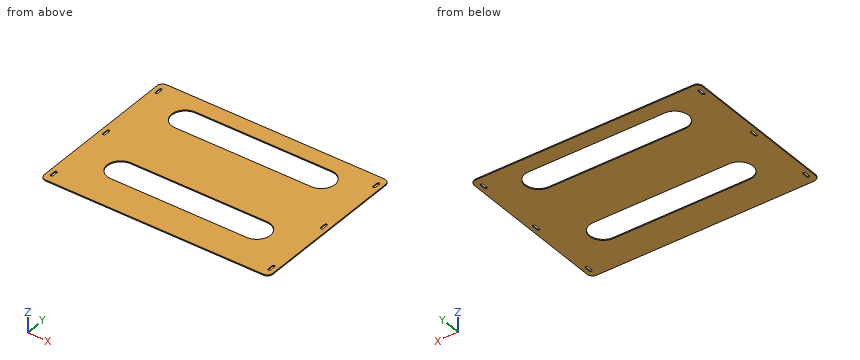
```python
from build123d import *

# Parameters (mm, degrees)
SKETCH_1_W          = 420
SKETCH_1_H          = 300
EXTRUDE_1_DEPTH     = 2
HOLE_WIZARD_M4_2_D  = 3.3
CUT_EXTRUDE_1_DEPTH = 10
FILLET_1_R          = 10
CUT_EXTRUDE_2_DEPTH = 10


with BuildPart() as part:
    # 草图1 → 凸台-拉伸1 (new body)
    with BuildSketch(Plane.XY):
        Rectangle(SKETCH_1_W, SKETCH_1_H)
    extrude(amount=EXTRUDE_1_DEPTH)

    # M4 螺纹孔的螺纹孔钻头2 (through all)
    with Locations(Plane.XY.offset(2)):
        with Locations((200, 0), (-200, -130), (-200, 0), (200, -130)):
            Hole(HOLE_WIZARD_M4_2_D / 2)

    # 草图4 → 切除-拉伸1 (cut)
    with BuildSketch(Plane.XY.offset(2)):
        with BuildLine():
            Line((197.75, -135), (197.75, -125))
            ThreePointArc((197.75, -125), (200, -122.75), (202.25, -125))
            Line((202.25, -125), (202.25, -135))
            ThreePointArc((202.25, -135), (200, -137.25), (197.75, -135))
        make_face()
        with BuildLine():
            Line((-197.75, -135), (-197.75, -125))
            ThreePointArc((-197.75, -125), (-200, -122.75), (-202.25, -125))
            Line((-202.25, -125), (-202.25, -135))
            ThreePointArc((-202.25, -135), (-200, -137.25), (-197.75, -135))
        make_face()
        with BuildLine():
            Line((202.25, -5), (202.25, 5))
            ThreePointArc((202.25, 5), (200, 7.25), (197.75, 5))
            Line((197.75, 5), (197.75, -5))
            ThreePointArc((197.75, -5), (200, -7.25), (202.25, -5))
        make_face()
        with BuildLine():
            Line((197.75, 135), (197.75, 125))
            ThreePointArc((197.75, 125), (200, 122.75), (202.25, 125))
            Line((202.25, 125), (202.25, 135))
            ThreePointArc((202.25, 135), (200, 137.25), (197.75, 135))
        make_face()
        with BuildLine():
            Line((-197.75, 135), (-197.75, 125))
            ThreePointArc((-197.75, 125), (-200, 122.75), (-202.25, 125))
            Line((-202.25, 125), (-202.25, 135))
            ThreePointArc((-202.25, 135), (-200, 137.25), (-197.75, 135))
        make_face()
        with BuildLine():
            Line((-202.25, -5), (-202.25, 5))
            ThreePointArc((-202.25, 5), (-200, 7.25), (-197.75, 5))
            Line((-197.75, 5), (-197.75, -5))
            ThreePointArc((-197.75, -5), (-200, -7.25), (-202.25, -5))
        make_face()
    extrude(amount=-CUT_EXTRUDE_1_DEPTH, mode=Mode.SUBTRACT)

    # 圆角1
    fillet_1_edges = [part.edges().sort_by_distance(p)[0] for p in [
        (210, -150, 1),
        (-210, -150, 1),
        (-210, 150, 1),
        (210, 150, 1),
    ]]
    fillet(fillet_1_edges, radius=FILLET_1_R)

    # 草图5 → 切除-拉伸2 (cut)
    with BuildSketch(Plane.XY.offset(2)):
        with BuildLine():
            Line((-125, -40), (125, -40))
            ThreePointArc((125, -40), (150, -65), (125, -90))
            Line((125, -90), (-125, -90))
            ThreePointArc((-125, -90), (-150, -65), (-125, -40))
        make_face()
        with BuildLine():
            Line((125, 70), (-125, 70))
            ThreePointArc((-125, 70), (-150, 95), (-125, 120))
            Line((-125, 120), (125, 120))
            ThreePointArc((125, 120), (150, 95), (125, 70))
        make_face()
    extrude(amount=-CUT_EXTRUDE_2_DEPTH, mode=Mode.SUBTRACT)


solid = part.part
```
Verification items for the finished model (mm, model axes). Round coordinates to 2 decimals unless told otherwise and drop trailing zeros. Write each loop counter-clockwise with the first axis right and the second up, starting at its lowest first coordinate (ties: lowest second). Pieces come first, ordered by that corner, then holes. Notation, with made-up numbers: (-1, -12.75) -> (13, -12.75) arc R20 ccw to (13, 17.25) -> close; hole circle Ø11 at (-6, -7). An arc over 180 degrees is marked (long way). Write each question's results on one line, items separated by ' | '. Start each with the question number.
1. Cross-section at A-A (x = -101.5). Enter the section's corners in (y, z).
2. Cross-section at D-D (y = 114). Enter the section's corners in (x, z), then the cut area to 3 significant figures.
3. Material ranges on probe 1 along Y at (x, z) = (-30, 1.4); probe 2 along X at (y, z) = (126.5, 0.5); probe 3 along Y at (x, z) = (136, 1.7), recorded low to high. Write a range as from..to.
4. Cross-section at C-C (z = 1.1). Count the separate pieces of the cut face and the enclosed holes in it, then the cut area to 3 significant figures.
5. Cross-section at B-B (y = -65). Enter the section's corners in (x, z).
Solutions:
1) outline: (-150, 0) -> (-90, 0) -> (-90, 2) -> (-150, 2) -> close; (-40, 0) -> (70, 0) -> (70, 2) -> (-40, 2) -> close; (120, 0) -> (150, 0) -> (150, 2) -> (120, 2) -> close
2) outline: (-210, 0) -> (-141.25, 0) -> (-141.25, 2) -> (-210, 2) -> close; (141.25, 0) -> (210, 0) -> (210, 2) -> (141.25, 2) -> close | area: 275 mm2
3) probe 1: y = -150..-90, -40..70, 120..150 | probe 2: x = -210..-202.25, -197.75..197.75, 202.25..210 | probe 3: y = -150..-87.45, -42.55..72.55, 117.45..150
4) separate pieces: 1 | enclosed holes: 8 | area: 96,600 mm2
5) outline: (-210, 0) -> (-150, 0) -> (-150, 2) -> (-210, 2) -> close; (150, 0) -> (210, 0) -> (210, 2) -> (150, 2) -> close
